Geometry check sheet. Reference: the model listing, model coordinates, mm. Coordinates: 2 decimals unless noted, no trailing zeros. Write each loop counter-clockwise with the first axis right and the second up, starting at its lowest first coordinate (ties: lowest second). Pieces come first, ordered by that corner, then holes. Notation, with made-up numbers: (-34, 71.25) -> (3, 71.25) arc R25 ccw to (3, 93.25) -> close; hole circle Ø6 at (-4.75, 42.5). An arc over 180 degrees is marked (long way). Answer in a Markdown table with one row per item. Add a question column.
1. Scan lines: L1, parallel to X at y = 7.5, z = -50; L2, parallel to Z at x = -25, y = 12.25; L3, parallel to X at y = 11.75, z = 53. Record each from-to range of solid material in increasing order. Write a range as from..to.
2. Cross-section at C-C on y = 19.5. Record the cut outline in (x, z), and give its area (3 significant figures).
3. Cross-section at B-B on z = 50. Record the cut outline in (x, y), and give its area (3 significant figures).
4. Cross-section at A-A on x = 25. Record the cut outline in (y, z).
5. Depth check by flat-ended pin: P1, Ø5.5, axis at x = -25, z = -50, coming from the +Y side. Enter the tip coordinate at first touch or a pass-through.
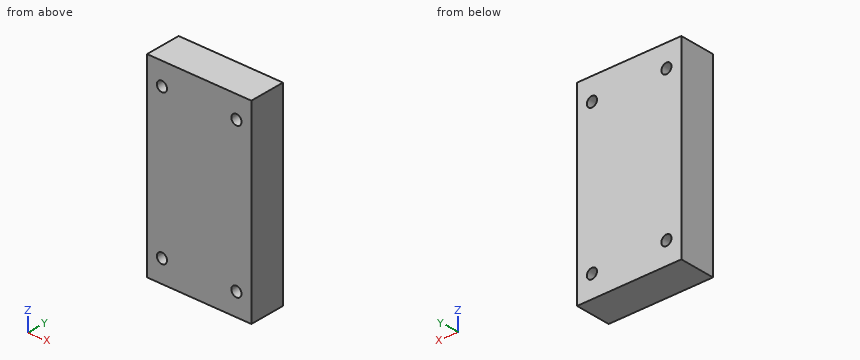
```python
from build123d import *

# Parameters (mm, degrees)
SKETCH_1_W         = 70
SKETCH_1_H         = 130
EXTRUDE_1_DEPTH    = 24
HOLE_WIZARD_M8_1_D = 6.8


with BuildPart() as part:
    # 草图1 → 凸台-拉伸1 (new body)
    with BuildSketch(Plane(origin=(0, 0, 0), x_dir=(1, 0, 0), z_dir=(0, 1, 0))):
        Rectangle(SKETCH_1_W, SKETCH_1_H)
    extrude(amount=EXTRUDE_1_DEPTH)

    # M8 螺纹孔1 (through all)
    with Locations(Plane(origin=(0, 24, 0), x_dir=(1, 0, 0), z_dir=(0, 1, 0))):
        with Locations((-25, -50), (-25, 50), (25, 50), (25, -50)):
            Hole(HOLE_WIZARD_M8_1_D / 2)


solid = part.part
```
Results found:
| question | item | result |
|---|---|---|
| 1 | L1 | x = -35..-28.4, -21.6..21.6, 28.4..35 |
| 1 | L2 | z = -65..-53.4, -46.6..46.6, 53.4..65 |
| 1 | L3 | x = -35..-26.6, -23.4..23.4, 26.6..35 |
| 2 | outline | (-35, -65) -> (35, -65) -> (35, 65) -> (-35, 65) -> close; hole circle Ø6.8 at (-25, -50); hole circle Ø6.8 at (-25, 50); hole circle Ø6.8 at (25, -50); hole circle Ø6.8 at (25, 50) |
| 2 | area | 8,950 mm^2 |
| 3 | outline | (-35, 0) -> (-28.4, 0) -> (-28.4, 24) -> (-35, 24) -> close; (-21.6, 0) -> (21.6, 0) -> (21.6, 24) -> (-21.6, 24) -> close; (28.4, 0) -> (35, 0) -> (35, 24) -> (28.4, 24) -> close |
| 3 | area | 1,350 mm^2 |
| 4 | outline | (0, -65) -> (24, -65) -> (24, -53.4) -> (0, -53.4) -> close; (0, -46.6) -> (24, -46.6) -> (24, 46.6) -> (0, 46.6) -> close; (0, 53.4) -> (24, 53.4) -> (24, 65) -> (0, 65) -> close |
| 5 | P1 | passes through |
